from build123d import *

# Parameters (mm, degrees)
SKETCH1_R           = 0.625
BOSS_EXTRUDE2_DEPTH = 1.5
SKETCH3_R           = 0.75
SKETCH3_R_2         = 0.4
CUT_EXTRUDE1_DEPTH  = 0.5
FILLET1_R           = 2


with BuildPart() as part:
    # Sketch1 → Boss-Extrude2 (new body)
    with BuildSketch(Plane.XY):
        with BuildLine():
            Line((0, 0), (20, 0))
            ThreePointArc((20, 0), (21, -1), (20, -2))
            Line((20, -2), (-1.154700538, -2))
            Line((-1.154700538, -2), (0, 0))
        make_face()
        with Locations((20, -1)):
            Circle(SKETCH1_R, mode=Mode.SUBTRACT)
    extrude(amount=BOSS_EXTRUDE2_DEPTH)

    # Sketch3 → Cut-Extrude1 (cut, symmetric)
    # profile 1 of 5: a face of its own
    with BuildSketch(Plane(origin=(0, 0, 0.75), x_dir=(-1, 0, 0), z_dir=(0, 0, -1))):
        with BuildLine():
            ThreePointArc((-1.371206885, -0.874999993), (-1.096687833, -0.600480945), (-0.721687836, -0.5))
            Line((-0.721687836, -0.5), (-1.154700538, -0.5))
            Line((-1.154700538, -0.5), (-1.371206885, -0.874999993))
        make_face()
    # profile 2 of 5: a face of its own
    with BuildSketch(Plane(origin=(0, 0, 0.75), x_dir=(-1, 0, 0), z_dir=(0, 0, -1))):
        with BuildLine():
            ThreePointArc((-0.721687836, -0.5), (-0.346687831, -0.60048095), (-0.072168777, -0.875000011))
            Line((-0.072168777, -0.875000011), (-0.288675135, -0.5))
            Line((-0.288675135, -0.5), (-0.721687836, -0.5))
        make_face()
    # profile 3 of 5: a face of its own
    with BuildSketch(Plane(origin=(0, 0, 0.75), x_dir=(-1, 0, 0), z_dir=(0, 0, -1))):
        with BuildLine():
            Line((-0.721687836, -2), (0.577350269, -2))
            Line((0.577350269, -2), (-0.072168777, -0.875000011))
            ThreePointArc((-0.072168777, -0.875000011), (0.002756535, -1.055885722), (0.028312164, -1.25))
            ThreePointArc((0.028312164, -1.25), (-0.191357751, -1.780330086), (-0.721687836, -2))
        make_face()
    # profile 4 of 5: a face of its own
    with BuildSketch(Plane(origin=(0, 0, 0.75), x_dir=(-1, 0, 0), z_dir=(0, 0, -1))):
        with BuildLine():
            Line((-2.020725942, -2), (-0.721687836, -2))
            ThreePointArc((-0.721687836, -2), (-1.371206891, -1.624999997), (-1.371206885, -0.874999993))
            Line((-1.371206885, -0.874999993), (-2.020725942, -2))
        make_face()
    # profile 5 of 5: a face of its own
    with BuildSketch(Plane(origin=(0, 0, 0.75), x_dir=(-1, 0, 0), z_dir=(0, 0, -1))):
        with Locations((-0.721687836, -1.25)):
            Circle(SKETCH3_R)
        with Locations((-0.721687836, -1.25)):
            Circle(SKETCH3_R_2, mode=Mode.SUBTRACT)
    extrude(amount=CUT_EXTRUDE1_DEPTH, both=True, mode=Mode.SUBTRACT)

    # Fillet1
    fillet1_edges = [part.edges().sort_by_distance(p)[0] for p in [
        (0, 0, 0.75),
    ]]
    fillet(fillet1_edges, radius=FILLET1_R)


solid = part.part
Could you check a few things on this model? Use its own coordinates, in mm. A direction names the side the tool comes from. Round coordinates to 2 decimals unless told otherwise and drop trailing zeros. Write each loop counter-clockwise with the first axis right and the second up, starting at its lowest first coordinate (ties: lowest second). Pieces come first, ordered by that corner, then holes. Notation, with made-up numbers: (-31, -30) - (25, -30) arc R28 ccw to (25, -6) - close; hole circle Ø4 at (-33, 27.25). An arc over 180 degrees is marked (long way). Put each result on its own line as item: value. Start each with the question number.
(1) I need wall thicknesses on probe 1 along X at (y, z) = (-0.75, 1); probe 2 along X at (y, z) = (-0.7, 1.05); probe 3 along Y at (x, z) = (20, 1) (3 decimals). Which ranges of each line are inside material? Lowest first, please.
(2) Thinking about a two-plate mould opening in X: for faces 1 (the flat face through (0.45, -1.74, 1.25)), 2 (the flat face through (10, 0, 1)), 3 (the cylindrical face through (0.17, -0.26, 0.76)), 4 (the cylindrical face through (19.376, -0.973, 0.74)), which applies, released by +X, released by -X, zero draft, split by the parting line, or undercut?
(3) I want a section at C-C, the plane x = 19.75. Please give me the cut outline in (y, z).
(4) I want a section at A-A, the plane z = 0.8. Please give me the cut outline in (x, y) (3 decimals), plus the area to 3 significant figures.
(5) For faces 5 (the flat face through (1, -0.5, 1)), 6 (the flat face through (10, -1, 1.5)), which set-ups out of +Z, -Z, +X, -X, +Y, -Y let a thin tool reach every point of the face, with its end or its side?
(6) I want a section at B-B, the plane y = -1.25. Please give me the cut outline in (x, z).
Here are the results:
1. probe 1: x = -0.41 to 0.14, 1.3 to 19.43, 20.57 to 20.97
1. probe 2: x = -0.37 to 0.17, 1.27 to 19.45, 20.55 to 20.95
1. probe 3: y = -2 to -1.625, -0.375 to 0
2. face 1: undercut
2. face 2: zero draft
2. face 3: released by -X
2. face 4: undercut
3. outline: (-2, 0) - (-1.57, 0) - (-1.57, 1.5) - (-2, 1.5) - close; (-0.43, 0) - (0, 0) - (0, 1.5) - (-0.43, 1.5) - close
4. outline: (-1.155, -2) - (-0.577, -2) - (0.289, -0.5) - (1.155, -0.5) - (2.021, -2) - (20, -2) arc R1 ccw to (20, 0) - (1.155, 0) arc R2 ccw to (-0.577, -1) - close; circle Ø0.8 at (0.722, -1.25); hole circle Ø1.25 at (20, -1)
4. area: 39.2 mm^2
5. face 5: none
5. face 6: +Z, +X, -X, +Y, -Y
6. outline: (-0.72, 0) - (19.43, 0) - (19.43, 1.5) - (-0.72, 1.5) - close; (20.57, 0) - (20.97, 0) - (20.97, 1.5) - (20.57, 1.5) - close; hole (-0.14, 0.25) - (0.32, 0.25) - (0.32, 1.25) - (-0.14, 1.25) - close; hole (1.12, 0.25) - (1.59, 0.25) - (1.59, 1.25) - (1.12, 1.25) - close
